```python
from build123d import *

# Parameters (mm, degrees)
SKETCH_1_R          = 130
SKETCH_1_R_2        = 10
EXTRUDE_1_DEPTH     = 10
SKETCH_2_R          = 55
EXTRUDE_2_DEPTH     = 20
SKETCH_3_R          = 45
CUT_EXTRUDE_1_DEPTH = 20
CHAMFER_1_SIZE      = 10


with BuildPart() as part:
    # 草图1 → 凸台-拉伸1 (new body)
    with BuildSketch(Plane.XY):
        Circle(SKETCH_1_R)
        with Locations((0, 108)):
            Circle(SKETCH_1_R_2, mode=Mode.SUBTRACT)
        with Locations((76.367532368, 76.367532368)):
            Circle(SKETCH_1_R_2, mode=Mode.SUBTRACT)
        with Locations((108, 0)):
            Circle(SKETCH_1_R_2, mode=Mode.SUBTRACT)
        with Locations((76.367532368, -76.367532368)):
            Circle(SKETCH_1_R_2, mode=Mode.SUBTRACT)
        with Locations((0, -108)):
            Circle(SKETCH_1_R_2, mode=Mode.SUBTRACT)
        with Locations((-76.367532368, -76.367532368)):
            Circle(SKETCH_1_R_2, mode=Mode.SUBTRACT)
        with Locations((-108, 0)):
            Circle(SKETCH_1_R_2, mode=Mode.SUBTRACT)
        with Locations((-76.367532368, 76.367532368)):
            Circle(SKETCH_1_R_2, mode=Mode.SUBTRACT)
    extrude(amount=EXTRUDE_1_DEPTH)

    # 草图2 → 凸台-拉伸2 (add)
    with BuildSketch(Plane.XY.offset(10)):
        Circle(SKETCH_2_R)
    extrude(amount=EXTRUDE_2_DEPTH)

    # 草图3 → 切除-拉伸1 (cut)
    with BuildSketch(Plane(origin=(0, 0, 0), x_dir=(-1, 0, 0), z_dir=(0, 0, -1))):
        Circle(SKETCH_3_R)
    extrude(amount=-CUT_EXTRUDE_1_DEPTH, mode=Mode.SUBTRACT)

    # 倒角1
    chamfer_1_edges = [part.edges().sort_by_distance(p)[0] for p in [
        (-55, 0, 30),
    ]]
    chamfer(chamfer_1_edges, length=CHAMFER_1_SIZE)


solid = part.part
```
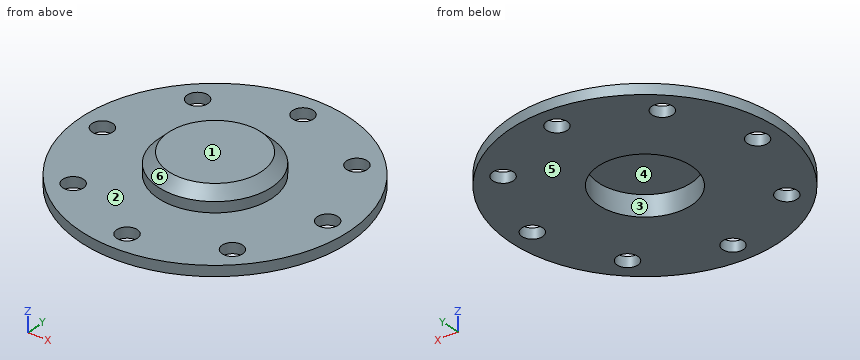
Design review of the part built by this model. Coordinates are the model's own, in mm. Face numbers are marked on the shaded views. A direction names the side the tool comes from. Coordinates: 2 decimals unless noted, no trailing zeros. Loops run counter-clockwise (first coordinate to the right, second up) from the corner with the lowest first, then second, coordinate; pieces in that order, holes last. Notation, with made-up numbers: (3, -12.75) -> (33, -12.75) arc R23 ccw to (33, -3.75) -> close; hole circle Ø11 at (34.25, 18). An arc over 180 degrees is marked (long way). Answer as a JSON object with one key per item and string values.
Q1. To check wall thickness, follow L1, parallel to Y at x = 0, z = 3.75; L2, parallel to X at y = 0.5, z = 6.25; L3, parallel to Z at x = 32, y = 97.5. State the ranges of each line that lie inside material, in increasing order.
Answer block:
{"L1": "y = -130 to -118, -98 to -45, 45 to 98, 118 to 130", "L2": "x = -130 to -117.99, -98.01 to -45, 45 to 98.01, 117.99 to 130", "L3": "z = 0 to 10"}
Q2. Take a section at C-C on z = 5. Give the number of separate pieces and of enclosed holes in the cut face, plus the area to 3 significant figures.
Answer block:
{"separate pieces": "1", "enclosed holes": "9", "area": "44,200 mm^2"}
Q3. Tool access review of the marked faces 1, 2 and 3: name each direction out of +Z, -Z, +X, -X, +Y, -Y from which nothing blocks a thin tool from reaching the whole face with its end or side.
Answer block:
{"face 1": "+Z, +X, -X, +Y, -Y", "face 2": "+Z", "face 3": "-Z"}
Q4. Take a section at D-D on x = -108. Give the boundary of the cut face in (y, z).
Answer block:
{"outline": "(-72.36, 0) -> (-10, 0) -> (-10, 10) -> (-72.36, 10) -> close; (10, 0) -> (72.36, 0) -> (72.36, 10) -> (10, 10) -> close"}
Q5. Clearance check with flat-ended pins moving along their axes: pin 1 Ø12 at (x, y) = (76.37, -76.37) entering from -Z; pin 2 Ø12 at (y, z) = (-49.5, 14) entering from -X; pin 3 Ø1.5 at (x, z) = (-22, 6.5) entering from +Y; pin 4 Ø12 at (y, z) = (21.5, 18.5) entering from -X. State where each tip first meets the part, or that it passes through.
Answer block:
{"pin 1": "passes through", "pin 2": "stops at x = -121.95", "pin 3": "stops at y = 128.25", "pin 4": "stops at x = -52.77"}
Q6. Take a section at A-A on x = 0. Give the boundary of the cut face in (y, z).
Answer block:
{"outline": "(-130, 0) -> (-118, 0) -> (-118, 10) -> (-130, 10) -> close; (-98, 0) -> (-45, 0) -> (-45, 20) -> (45, 20) -> (45, 0) -> (98, 0) -> (98, 10) -> (55, 10) -> (55, 20) -> (45, 30) -> (-45, 30) -> (-55, 20) -> (-55, 10) -> (-98, 10) -> close; (118, 0) -> (130, 0) -> (130, 10) -> (118, 10) -> close"}
Q7. The part is to be moulded in two halves that separate along Y. For the marked faces 4, 5 and 6, say which applies: +Y half, -Y half, draft (parallel to the pull), parting line (faces both ways), or undercut.
Answer block:
{"face 4": "undercut", "face 5": "draft", "face 6": "parting line"}
